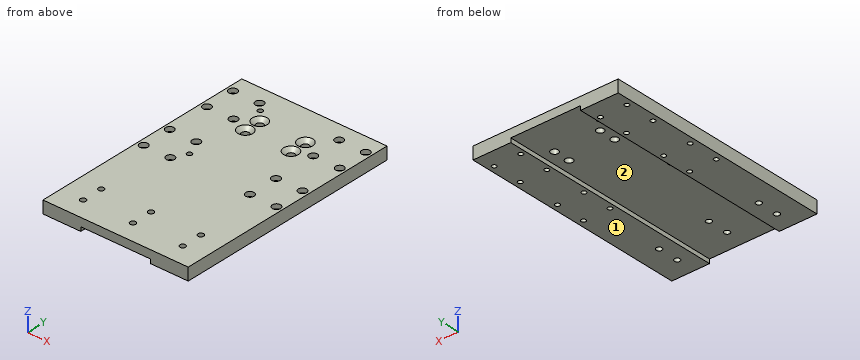
```python
from build123d import *

# Parameters (mm, degrees)
SKETCH_1_W                   = 175
SKETCH_1_H                   = 275
EXTRUDE_1_DEPTH              = 10
SKETCH_10_W                  = 45.5
SKETCH_10_H                  = 275
EXTRUDE_2_DEPTH              = 5
HOLE_WIZARD_M8_1_D           = 9
HOLE_WIZARD_M8_1_CSINK_D     = 17.92
HOLE_WIZARD_M8_1_CSINK_ANGLE = 90
HOLE_WIZARD_M8_1_2_D         = 6.8
HOLE_WIZARD_M5_1_D           = 5.5
HOLE_WIZARD_M5_1_CBORE_D     = 10
HOLE_WIZARD_M5_1_CBORE_DEPTH = 5.4
F_6_0MM_1_D                  = 6


with BuildPart() as part:
    # 草图1 → 凸台-拉伸1 (new body)
    with BuildSketch(Plane.XY):
        Rectangle(SKETCH_1_W, SKETCH_1_H)
    extrude(amount=EXTRUDE_1_DEPTH)

    # 草图10 → 凸台-拉伸2 (add)
    with BuildSketch(Plane(origin=(0, 0, 0), x_dir=(-1, 0, 0), z_dir=(0, 0, -1))):
        with Locations((-64.75, 0)):
            Rectangle(SKETCH_10_W, SKETCH_10_H)
        with Locations((64.75, 0)):
            Rectangle(SKETCH_10_W, SKETCH_10_H)
    extrude(amount=EXTRUDE_2_DEPTH)

    # Hole Wizard M8 _1 (through all)
    with Locations(Plane.XY.offset(10)):
        with Locations((-27.5, 93.5), (-27.5, 73.5), (27.5, 93.5), (27.5, 73.5)):
            CounterSinkHole(HOLE_WIZARD_M8_1_D / 2, HOLE_WIZARD_M8_1_CSINK_D / 2, counter_sink_angle=HOLE_WIZARD_M8_1_CSINK_ANGLE)

    # Hole Wizard M8 _1 2 (through all)
    with Locations(Plane.XY.offset(10)):
        with Locations((0, -113.5), (-60, -113.5), (60, -113.5), (0, -88.5), (-60, -88.5), (60, -88.5)):
            Hole(HOLE_WIZARD_M8_1_2_D / 2)

    # M5 六角凹头螺钉的柱形沉头孔1 (through all)
    with Locations(Plane.XY.offset(10)):
        with Locations((-80, 116.75), (-48, 116.75), (-80, 80.75), (-48, 80.75), (-80, 29.25), (-48, 29.25), (-80, -6.75), (-48, -6.75), (48, -6.75), (80, -6.75), (48, 29.25), (80, 29.25), (48, 80.75), (80, 80.75), (48, 116.75), (80, 116.75)):
            CounterBoreHole(HOLE_WIZARD_M5_1_D / 2, HOLE_WIZARD_M5_1_CBORE_D / 2, HOLE_WIZARD_M5_1_CBORE_DEPTH)

    # Ø6.0mm 暗销孔1 (through all)
    with Locations(Plane.XY.offset(10)):
        with Locations((-39, 107.5), (-39, 9.5)):
            Hole(F_6_0MM_1_D / 2)


solid = part.part
```
Verification items for the finished model (mm, model axes). Face numbers are marked on the shaded views. Round coordinates to 2 decimals unless told otherwise and drop trailing zeros. Order: outer loops, then holes, each group sorted by start corner. A loop starts at its lowest first (then second) coordinate and runs counter-clockwise, first axis right, second up. Notation, with made-up numbers: (77, 28.25) - (91, 28.25) arc R13 cw to (91, 37.25) - close; hole circle Ø1 at (-31.5, 4.5). An arc over 180 degrees is marked (long way). Use CSV: the item, a comma, the result in double quotes. Start each with the question number.
1) Section check B-B, the plane y = -88.5. Record the cut outline in (x, z).
2) Mould release check, pull along X, two halves, no side actions. Record for the marked faces 1 and 2: +X half, -X half, draft (parallel to the pull), parting line (faces both ways), or undercut.
3) Section check D-D, the plane x = -80. State how many separate pieces and enclosed holes the cut face has, plus the area to 3 significant figures.
4) Go/stop test with flat-tipped pins: P1, Ø14.5, axis at x = -27.5, y = 93.5, coming from the -Z side; P2, Ø6.5, axis at x = -80, y = 29.25, coming from the +Z side. Record where each tip stops, or that it passes through.
5) Section check A-A, the plane x = 0. Record the cut outline in (y, z).
6) Section check C-C, the plane y = 93.5. Record the cut outline in (x, z).
7) Thickness scan on L1, parallel to X at y = 81, z = 5.5; L2, parallel to Y at x = 48, z = -1.5; L3, parallel to Y at x = -80, z = 8.6. Record the ranges inside material, lowest first.
Answers:
1,outline,"(-87.5, -5) - (-63.4, -5) - (-63.4, 10) - (-87.5, 10) - close; (-56.6, -5) - (-42, -5) - (-42, 0) - (-3.4, 0) - (-3.4, 10) - (-56.6, 10) - close; (3.4, 0) - (42, 0) - (42, -5) - (56.6, -5) - (56.6, 10) - (3.4, 10) - close; (63.4, -5) - (87.5, -5) - (87.5, 10) - (63.4, 10) - close"
2,face 1,"draft"
2,face 2,"undercut"
3,separate pieces,"5"
3,enclosed holes,"0"
3,area,"3,700 mm²"
4,P1,"stops at z = 0"
4,P2,"stops at z = 4.6"
5,outline,"(-137.5, 0) - (-116.9, 0) - (-116.9, 10) - (-137.5, 10) - close; (-110.1, 0) - (-91.9, 0) - (-91.9, 10) - (-110.1, 10) - close; (-85.1, 0) - (137.5, 0) - (137.5, 10) - (-85.1, 10) - close"
6,outline,"(-87.5, -5) - (-42, -5) - (-42, 0) - (-32, 0) - (-32, 5.54) - (-36.46, 10) - (-87.5, 10) - close; (-23, 0) - (23, 0) - (23, 5.54) - (18.54, 10) - (-18.54, 10) - (-23, 5.54) - close; (32, 0) - (42, 0) - (42, -5) - (87.5, -5) - (87.5, 10) - (36.46, 10) - (32, 5.54) - close"
7,L1,"x = -87.5 to -84.99, -75.01 to -52.99, -43.01 to 43.01, 52.99 to 75.01, 84.99 to 87.5"
7,L2,"y = -137.5 to -9.5, -4 to 26.5, 32 to 78, 83.5 to 114, 119.5 to 137.5"
7,L3,"y = -137.5 to -11.75, -1.75 to 24.25, 34.25 to 75.75, 85.75 to 111.75, 121.75 to 137.5"
